Verification items for the finished model (mm, model axes). A direction names the side the tool comes from. Give positions to 0.01 mm unless a question says otherwise; leave off trailing zeros. Write each loop counter-clockwise with the first axis right and the second up, starting at its lowest first coordinate (ties: lowest second). Pieces come first, ordered by that corner, then holes.
from build123d import *

# Parameters (mm, degrees)
SHEET_EXTRUDE_1_1_BACK   = 45
SHEET_EXTRUDE_1_1_DEPTH  = 90
THICKEN_1_T2             = 3
EXTRUDE_START            = 42
EXTRUDE_3_DEPTH          = 3
CUT_EXTRUDE_1_DEPTH      = 811.963488807
CUT_EXTRUDE_1_DEPTH_BACK = 811.963488807
SKETCH_4_R               = 11
EXTRUDE_START_2          = 26.5
SKETCH_5_R               = 11
EXTRUDE_4_DEPTH          = 12


with BuildPart() as body_1:
    # Sheet Extrude 1: a surface, the sketch's curves swept straight by 90 mm
    with BuildLine(Plane.XY.offset(489.577688539).offset(-SHEET_EXTRUDE_1_1_BACK), mode=Mode.PRIVATE) as sheet_extrude_1_1_path:
        Line((-1467.361703007, 82), (-1467.361703007, 152))
        Line((-1467.361703007, 152), (-1317.361703007, 544.300904919))
        Line((-1317.361703007, 544.300904919), (-1067.361703007, 544.300904919))
        Line((-1067.361703007, 544.300904919), (-917.361703007, 152))
        Line((-917.361703007, 152), (-917.361703007, 82))
    sheet_extrude_1_1 = Shell.extrude(sheet_extrude_1_1_path.wire(), (0 * SHEET_EXTRUDE_1_1_DEPTH, 0 * SHEET_EXTRUDE_1_1_DEPTH, 1 * SHEET_EXTRUDE_1_1_DEPTH))
    add(Solid.thicken(sheet_extrude_1_1, -THICKEN_1_T2))

    # 草图3 → 凸台-拉伸3 (add)
    with BuildSketch(Plane.XY.offset(489.577688539).offset(EXTRUDE_START)):
        Polygon((-1464.361703007, 82), (-1434.361703007, 106.446018098), (-1434.361703007, 151.446018098), (-1296.767748095, 511.300904919), (-1192.361703007, 511.300904919), (-1192.361703007, 541.300904919), (-1315.296961402, 541.300904919), (-1464.361703007, 151.446018098), align=None)
    extrude(amount=EXTRUDE_3_DEPTH)

    # 镜向1: body 1 across plane


with BuildPart() as body_1_1:
    add(body_1.part)
    add(body_1.part.mirror(Plane.ZY.offset(1192.361703007)))

    # 镜向2: body 1 across plane


with BuildPart() as body_1_2:
    add(body_1_1.part)
    add(body_1_1.part.mirror(Plane.XY.offset(489.577688539)))

    # 草图4 → 切除-拉伸1 (cut, two sides: drawn at the far end of the back side and taken through both)
    with BuildSketch(Plane.ZY.offset(1192.361703007).offset(-CUT_EXTRUDE_1_DEPTH_BACK)):
        with Locations((489.577688539, 117)):
            Circle(SKETCH_4_R)
    extrude(amount=CUT_EXTRUDE_1_DEPTH + CUT_EXTRUDE_1_DEPTH_BACK, mode=Mode.SUBTRACT)

    # 草图5 → 凸台-拉伸4 (add)
    with BuildSketch(Plane.ZY.offset(1192.361703007).offset(EXTRUDE_START_2)):
        with BuildLine():
            Line((379.577688539, 621.300904919), (644.577688539, 621.300904919))
            ThreePointArc((644.577688539, 621.300904919), (651.64875635, 618.371972731), (654.577688539, 611.300904919))
            Line((654.577688539, 611.300904919), (654.577688539, 536.300904919))
            ThreePointArc((654.577688539, 536.300904919), (651.64875635, 529.229837107), (644.577688539, 526.300904919))
            Line((644.577688539, 526.300904919), (379.577688539, 526.300904919))
            ThreePointArc((379.577688539, 526.300904919), (372.506620727, 529.229837107), (369.577688539, 536.300904919))
            Line((369.577688539, 536.300904919), (369.577688539, 611.300904919))
            ThreePointArc((369.577688539, 611.300904919), (372.506620727, 618.371972731), (379.577688539, 621.300904919))
        make_face()
        with Locations((620.577688539, 587.300904919)):
            Circle(SKETCH_5_R, mode=Mode.SUBTRACT)
        with Locations((399.577688539, 571.300904919)):
            Circle(SKETCH_5_R, mode=Mode.SUBTRACT)
    extrude(amount=EXTRUDE_4_DEPTH)

    # 镜向3: body 1 across plane


with BuildPart() as body_1_3:
    add(body_1_2.part)
    add(body_1_2.part.mirror(Plane.ZY.offset(1192.361703007)))


solid = body_1_3.part
Item 1: Release check for a two-part mould opening along Z. For faces 1 (the face through (-1449.572, 94.052, 533.057)), 2 (the face through (-1230.862, 534, 490)) record: released by +Z, released by -Z, zero draft, split by the parting line, or undercut.
Answer key:
face 1: zero draft
face 2: undercut
Item 2: Scan lines: line 1 along Z through (x, y) = (-1077.5, 510); line 2 along Z through (x, y) = (-1465.1, 117); line 3 along X through (y, z) = (598, 503). Record each from-to range of solid material in increasing order.
Answer key:
line 1: z = 444.58 to 447.58, 531.58 to 534.58
line 2: z = 444.58 to 478.58, 500.58 to 534.58
line 3: x = -1230.86 to -1218.86, -1165.86 to -1153.86
Item 3: Depth check by flat-ended pin: pin 1 (10 mm diameter, centred on y = 461.5, z = 501, fed in from -X); pin 2 (4.5 mm diameter, centred on y = 533.5, z = 499, fed in from +X); pin 3 (16 mm diameter, centred on x = -1191, z = 507, fed in from -Y). Enter the tip coordinate at first touch or a pass-through.
Answer key:
pin 1: stops at x = -1350.93
pin 2: stops at x = -1062.37
pin 3: stops at y = 541.3
Item 4: Sectioned sample at A-A on y = 117. Record the cut outline in (x, z).
Answer key:
outline: (-1467.36, 444.58) - (-1434.36, 444.58) - (-1434.36, 447.58) - (-1464.36, 447.58) - (-1464.36, 478.58) - (-1467.36, 478.58) - close; (-1467.36, 500.58) - (-1464.36, 500.58) - (-1464.36, 531.58) - (-1434.36, 531.58) - (-1434.36, 534.58) - (-1467.36, 534.58) - close; (-950.36, 444.58) - (-917.36, 444.58) - (-917.36, 478.58) - (-920.36, 478.58) - (-920.36, 447.58) - (-950.36, 447.58) - close; (-950.36, 531.58) - (-920.36, 531.58) - (-920.36, 500.58) - (-917.36, 500.58) - (-917.36, 534.58) - (-950.36, 534.58) - close
Item 5: Sectioned sample at B-B on z = 587.5. Record the cut outline in (x, y), then the cut area to 3 significant figures.
Answer key:
outline: (-1230.86, 526.3) - (-1218.86, 526.3) - (-1218.86, 621.3) - (-1230.86, 621.3) - close; (-1165.86, 526.3) - (-1153.86, 526.3) - (-1153.86, 621.3) - (-1165.86, 621.3) - close
area: 2,280 mm2
Item 6: Set-up check for faces 3 (the face through (-1275, 544.301, 489)), 4 (the face through (-1050, 415, 447.578)), 5 (the face through (-1159.946, 580.576, 405.491)), 6 (the face through (-935.15, 94.05, 533.06)): record each of +Z, -Z, +X, -X, +Y, -Y from which the full face is reachable in a straight line by a thin tool's end or side.
Answer key:
face 3: +Z, -Z, -X, +Y
face 4: -Y
face 5: +X, -X
face 6: +Z, -Z, -Y
Item 7: Sectioned sample at C-C on y = 437.5. Record the cut outline in (x, z), then the cut area to 3 significant figures.
Answer key:
outline: (-1358.2, 444.58) - (-1324.99, 444.58) - (-1324.99, 447.58) - (-1354.99, 447.58) - (-1354.99, 531.58) - (-1324.99, 531.58) - (-1324.99, 534.58) - (-1358.2, 534.58) - close; (-1059.74, 444.58) - (-1026.53, 444.58) - (-1026.53, 534.58) - (-1059.74, 534.58) - (-1059.74, 531.58) - (-1029.74, 531.58) - (-1029.74, 447.58) - (-1059.74, 447.58) - close
area: 938 mm2
